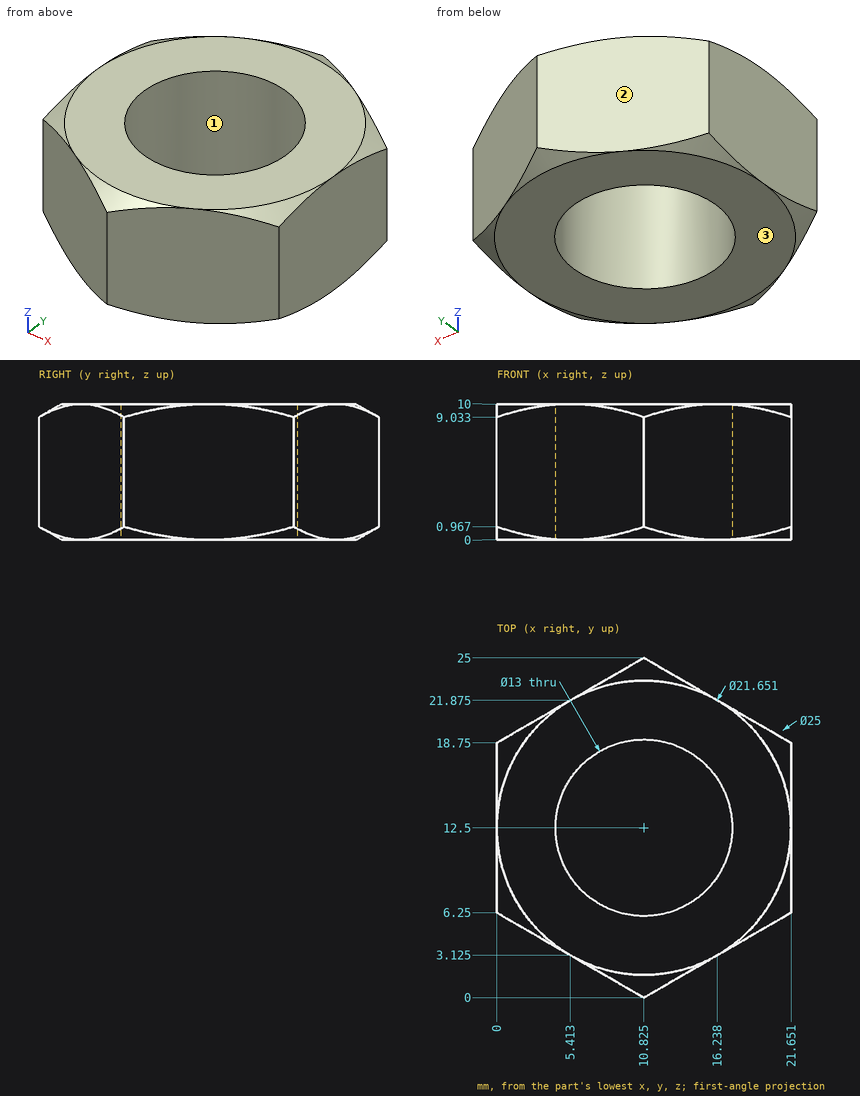
Input: dimensioned drawing with shaded views. Units: mm. Origin: part minimum x, y, z. Give positions to 0.01 mm unless a question says otherwise; leave off trailing zeros. One line per item, written item: value. Start each with the question number.
Q1. Material intervals for probe 1 along Y at (x, z) = (15.75, 7) (1 decimal); probe 2 along Y at (x, z) = (14.5, 7.25); probe 3 along X at (y, z) = (13.5, 6.25), sorted ascending. Write a range as from..to.
Q2. Draft query along X for the marked faces 1, 2 and 3. Return one class per face: +X half, -X half, draft (parallel to the pull), parting line (faces both ways), or undercut.
Q3. First-contact query: pin 1 Ø4 at (x, z) = (7, 7) entering from +Y; pin 2 Ø3 at (x, z) = (18, 7.5) entering from +Y; pin 3 Ø10.5 at (x, y) = (10.83, 12.5) entering from +Z; pin 4 Ø1 at (x, z) = (5.5, 5.5) entering from +Y (1 decimal). Flat tips, straight axial feed; report the tip coordinate or a pass-through.
Answer:
1. probe 1: y = 2.8..8.3, 16.7..22.2
1. probe 2: y = 2.12..7.14, 17.86..22.88
1. probe 3: x = 0..4.4, 17.25..21.65
2. face 1: undercut
2. face 2: -X half
2. face 3: draft
3. pin 1: stops at y = 23.95
3. pin 2: stops at y = 21.72
3. pin 3: passes through
3. pin 4: stops at y = 22.2
